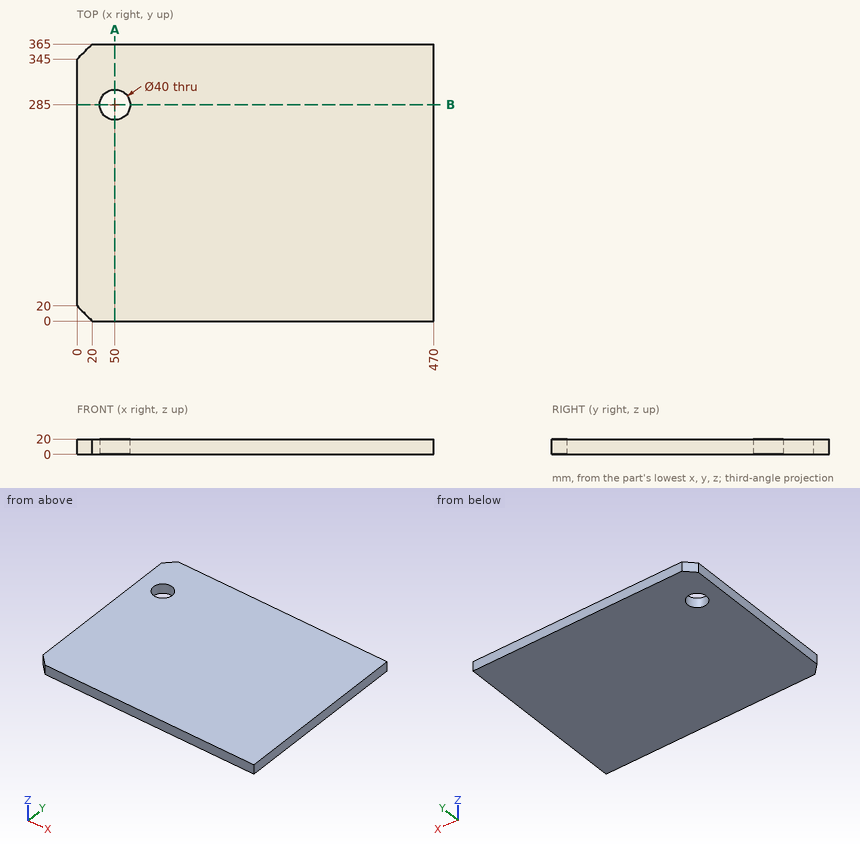
Design review of the part shown in the three views and the two pictorial views. Dimensions are in mm from the part's minimum x, y and z. Coordinates: 2 decimals unless noted, no trailing zeros. Order: outer loops, then holes, each group sorted by start corner. A loop starts at its lowest first (then second) coordinate and runs counter-clockwise, first axis right, second up.
1) Wall thickness on line 1 along X through (y, z) = (285, 6.5); line 2 along Y through (x, z) = (50, 14); line 3 along Y through (x, z) = (64.5, 7): over which ranges is each line inside the solid? List them lowest first.
2) Clearance check with a flat-ended pin moving along its axis: pin 1 (2 mm diameter, centred on y = 259.5, z = 2.5, fed in from -X). State where the tip first meets the part, or that it passes through.
3) Take a section at A-A, the plane x = 50. Give the boundary of the cut face in (y, z), and give its area (3 significant figures).
4) Take a section at B-B, the plane y = 285. Give the boundary of the cut face in (x, z), and give its area (3 significant figures).
Returned:
1. line 1: x = 0 to 30, 70 to 470
1. line 2: y = 0 to 265, 305 to 365
1. line 3: y = 0 to 271.23, 298.77 to 365
2. pin 1: stops at x = 0
3. outline: (0, 0) - (265, 0) - (265, 20) - (0, 20) - close; (305, 0) - (365, 0) - (365, 20) - (305, 20) - close
3. area: 6,500 mm2
4. outline: (0, 0) - (30, 0) - (30, 20) - (0, 20) - close; (70, 0) - (470, 0) - (470, 20) - (70, 20) - close
4. area: 8,600 mm2
